Design review of the part built by this model. Coordinates are the model's own, in mm. A direction names the side the tool comes from. Coordinates: 2 decimals unless noted, no trailing zeros. Loops run counter-clockwise (first coordinate to the right, second up) from the corner with the lowest first, then second, coordinate; pieces in that order, holes last. Notation, with made-up numbers: M 12.5,10 L 40.5,10 A24 ccw 40.5,36 Z; hole C 31,30.5 d11. An arc over 180 degrees is marked long. Put each result on its own line as item: value. Start each with the question number.
(1) Clearance check with flat-ended pins moving along their axes: pin 1 (1.8 mm diameter, centred on x = -1.5, y = -28.5, fed in from +Z); pin 2 (3 mm diameter, centred on x = -12, z = 0.5, fed in from +Y); pin 3 (3 mm diameter, centred on x = -23.5, z = 4, fed in from -Y). State where each tip first meets the part, or that it passes through.
(2) Take a section at B-B, the plane z = 4.35. Give the boundary of the cut face in (x, y).
(3) Take a section at A-A, the plane y = 0. Give the boundary of the cut face in (x, z).
(4) For probe 1 along Y at (x, z) = (-30, 3.5); probe 2 along Y at (x, z) = (-0.5, 5.7); probe 3 along X at (y, z) = (26.5, 2.45), list the stretches that pass through material, from the lowest coordinate up. Write a range as [from, to].
(5) For faces 1 (the flat face through (27, 0, 2)), 2 (the cylindrical face through (-0.867, -3.905, 3.042)), list the 3-axis set-ups (+Z, -Z, +X, -X, +Y, -Y) from which the entire face can be reached by the end or side of a thin tool; tool diameter is ignored.
(6) Take a section at C-C, the plane x = -27.5. Give the boundary of the cut face in (y, z), then the cut area to 3 significant figures.
(7) The part is to be moulded in two halves that separate along X. For faces 3 (the flat face through (7, 0, 0)), 4 (the cylindrical face through (18.28, 28.67, 2.96)), 5 (the cylindrical face through (24.5, 0.1, 4)), say which applies: +X half, -X half, draft (parallel to the pull), parting line (faces both ways), or undercut.
```python
from build123d import *

# Parameters (mm, degrees)
SKETCH1_R           = 34
BOSS_EXTRUDE1_DEPTH = 6
SKETCH2_R           = 3
CUT_EXTRUDE1_DEPTH  = 4
SKETCH3_R           = 4
CUT_EXTRUDE2_DEPTH  = 49.456165758


with BuildPart() as part:
    # Sketch1 → Boss-Extrude1 (new body)
    with BuildSketch(Plane.XY):
        Circle(SKETCH1_R)
    extrude(amount=BOSS_EXTRUDE1_DEPTH)

    # Sketch2 → Cut-Extrude1 (cut)
    with BuildSketch(Plane.XY.offset(6)):
        with Locations((0, 27.5)):
            Circle(SKETCH2_R)
        with Locations((27.5, 0)):
            Circle(SKETCH2_R)
        with Locations((0, -27.5)):
            Circle(SKETCH2_R)
        with Locations((-27.5, 0)):
            Circle(SKETCH2_R)
    extrude(amount=-CUT_EXTRUDE1_DEPTH, mode=Mode.SUBTRACT)

    # Sketch3 → Cut-Extrude2 (cut, through all)
    with BuildSketch(Plane.XY.offset(6)):
        Circle(SKETCH3_R)
    extrude(amount=-CUT_EXTRUDE2_DEPTH, mode=Mode.SUBTRACT)


solid = part.part
```
Computed values:
1. pin 1: stops at z = 2
1. pin 2: stops at y = 32.34
1. pin 3: stops at y = -25.92
2. outline: C 0,0 d68; hole C -27.5,0 d6; hole C 0,0 d8; hole C 0,-27.5 d6; hole C 0,27.5 d6; hole C 27.5,0 d6
3. outline: M -34,0 L -4,0 L -4,6 L -24.5,6 L -24.5,2 L -30.5,2 L -30.5,6 L -34,6 Z; M 4,0 L 34,0 L 34,6 L 30.5,6 L 30.5,2 L 24.5,2 L 24.5,6 L 4,6 Z
4. probe 1: y = [-16, -1.66], [1.66, 16]
4. probe 2: y = [-34, -30.46], [-24.54, -3.97], [3.97, 24.54], [30.46, 34]
4. probe 3: x = [-21.3, -2.83], [2.83, 21.3]
5. face 1: +Z
5. face 2: +Z, -Z
6. outline: M -19.99,0 L 19.99,0 L 19.99,6 L 3,6 L 3,2 L -3,2 L -3,6 L -19.99,6 Z
6. area: 216 mm^2
7. face 3: draft
7. face 4: parting line
7. face 5: undercut
